```python
from build123d import *

# Parameters (mm, degrees)
BASE_PLATE_SKETCH_W        = 100
BASE_PLATE_SKETCH_H        = 70
BASE_PLATE_100X70X12_DEPTH = 6
RAISED_PAD_SKETCH_W        = 94
RAISED_PAD_SKETCH_H        = 60
RAISED_PAD_94X60X4_DEPTH   = 4
PAD_CUT_1_DEPTH            = 2
PAD_CUT_2_DEPTH            = 2
PAD_CUT_3_DEPTH            = 2


with BuildPart() as part:
    # Base Plate Sketch → Base Plate 100x70x12 (new, symmetric)
    with BuildSketch(Plane.XY):
        Rectangle(BASE_PLATE_SKETCH_W, BASE_PLATE_SKETCH_H)
    extrude(amount=BASE_PLATE_100X70X12_DEPTH, both=True)

    # Raised Pad Sketch → Raised Pad 94x60x4 (add)
    with BuildSketch(Plane(origin=(0, 0, -6), x_dir=(-1, 0, 0), z_dir=(0, 0, -1))):
        Rectangle(RAISED_PAD_SKETCH_W, RAISED_PAD_SKETCH_H)
    extrude(amount=RAISED_PAD_94X60X4_DEPTH)

    # Pad Cut 1 Sketch → Pad Cut 1 (cut, symmetric)
    with BuildSketch(Plane(origin=(0, 0, -10), x_dir=(-1, 0, 0), z_dir=(0, 0, -1))):
        with BuildLine():
            Line((47, -23), (47, 23))
            Line((47, 23), (41, 23))
            ThreePointArc((41, 23), (37.464466094, 21.535533906), (36, 18))
            Line((36, 18), (36, 11.5))
            ThreePointArc((36, 11.5), (32.388712156, 0), (36, -11.5))
            Line((36, -11.5), (36, -18))
            ThreePointArc((36, -18), (37.464466094, -21.535533906), (41, -23))
            Line((41, -23), (47, -23))
        make_face()
    extrude(amount=PAD_CUT_1_DEPTH, both=True, mode=Mode.SUBTRACT)

    # Pad Cut 2 Sketch → Pad Cut 2 (cut, symmetric)
    with BuildSketch(Plane(origin=(0, 0, -10), x_dir=(-1, 0, 0), z_dir=(0, 0, -1))):
        with BuildLine():
            Line((-47, -6), (-39, -6))
            Line((-39, -6), (-39, -15))
            ThreePointArc((-39, -15), (-37.535533906, -18.535533906), (-34, -20))
            Line((-34, -20), (-30, -20))
            ThreePointArc((-30, -20), (-26.464466094, -18.535533906), (-25, -15))
            Line((-25, -15), (-25, -6))
            Line((-25, -6), (-22.017780858, -6.01060535))
            ThreePointArc((-22.017780858, -6.01060535), (-18.470758176, -4.552451776), (-17, -1.010636966))
            Line((-17, -1.010636966), (-17, 1))
            ThreePointArc((-17, 1), (-18.464466094, 4.535533906), (-22, 6))
            Line((-22, 6), (-25, 6))
            Line((-25, 6), (-25, 15))
            ThreePointArc((-25, 15), (-26.464466094, 18.535533906), (-30, 20))
            Line((-30, 20), (-34, 20))
            ThreePointArc((-34, 20), (-37.535533906, 18.535533906), (-39, 15))
            Line((-39, 15), (-39, 6))
            Line((-39, 6), (-47, 6))
            Line((-47, 6), (-47, -6))
        make_face()
    extrude(amount=PAD_CUT_2_DEPTH, both=True, mode=Mode.SUBTRACT)

    # Pad Cut 3 Sketch → Pad Cut 3 (cut, symmetric)
    with BuildSketch(Plane(origin=(0, 0, -10), x_dir=(-1, 0, 0), z_dir=(0, 0, -1))):
        with BuildLine():
            ThreePointArc((-10, 5.000015487), (-15.000015487, 0), (-10, -5.000015487))
            ThreePointArc((-10, -5.000015487), (-8.529332614, -8.524177957), (-5.000015487, -9.982431809))
            ThreePointArc((-5.000015487, -9.982431809), (0, -14.982447295), (5.000015487, -9.982431809))
            ThreePointArc((5.000015487, -9.982431809), (8.529332614, -8.524177957), (10, -5.000015487))
            ThreePointArc((10, -5.000015487), (15.000015487, 0), (10, 5.000015487))
            ThreePointArc((10, 5.000015487), (8.529332614, 8.524177957), (5.000015487, 9.982431809))
            ThreePointArc((5.000015487, 9.982431809), (0, 14.982447295), (-5.000015487, 9.982431809))
            ThreePointArc((-5.000015487, 9.982431809), (-8.529332614, 8.524177957), (-10, 5.000015487))
        make_face()
    extrude(amount=PAD_CUT_3_DEPTH, both=True, mode=Mode.SUBTRACT)


solid = part.part
```
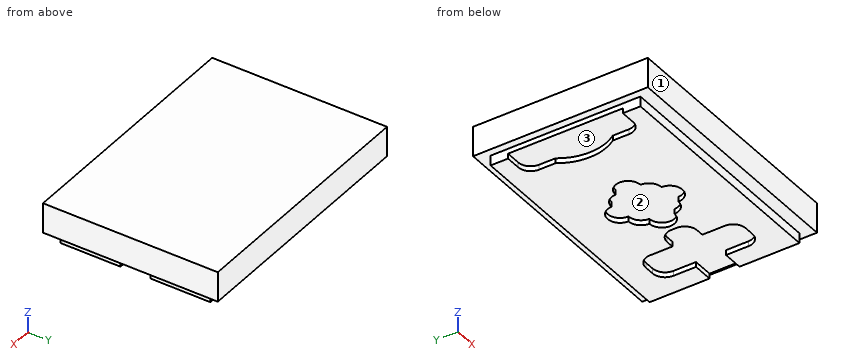
Verification items for the finished model (mm, model axes). Face numbers are marked on the shaded views. A direction names the side the tool comes from. Give positions to 0.01 mm unless a question says otherwise; leave off trailing zeros. Loops run counter-clockwise (first coordinate to the right, second up) from the corner with the lowest first, then second, coordinate; pieces in that order, holes last. Notation, with made-up numbers: M -39,-33.5 L -31,-33.5 A26 cw -31,3.5 Z; hole C -33,18.25 d3. An arc over 180 degrees is marked long. One line per question, with ' | ' between items.
Item 1: Thickness scan on line 1 (Y direction, x = 33, z = -8.25); line 2 (Z direction, x = -46, y = -19); line 3 (X direction, y = 11, z = -6.25). Record the ranges inside material, lowest first. Write a range as [from, to].
Completed:
line 1: y = [-30, -20], [20, 30] | line 2: z = [-8, 6] | line 3: x = [-47, 47]
Item 2: Depth check by flat-ended pin: P1, Ø2, axis at y = -9.5, z = -8.5, coming from the +X side; P2, Ø1.6, axis at x = 33, z = -9.5, coming from the +Y side; P3, Ø1.6, axis at x = 44.5, z = -9, coming from the -Y side. Enter the tip coordinate at first touch or a pass-through.
Completed:
P1: stops at x = 47 | P2: stops at y = 30 | P3: stops at y = -30
Item 3: Section check D-D, the plane x = 19. Record the cut outline in (y, z).
Completed:
outline: M -35,-6 L -30,-6 L -30,-10 L -5.01,-10 L -5.01,-8 L 5,-8 L 5,-10 L 30,-10 L 30,-6 L 35,-6 L 35,6 L -35,6 Z
Item 4: Section check A-A, the plane y = 28. Record the cut outline in (x, z).
Completed:
outline: M -50,-6 L -47,-6 L -47,-10 L 47,-10 L 47,-6 L 50,-6 L 50,6 L -50,6 Z
Item 5: Tool access check on the marked faces 1, 2 and 3. Record the directions out of +Z, -Z, +X, -X, +Y, -Y that give a thin tool (end or side, any length) a straight path to the whole face; none if there is none.
Completed:
face 1: +Z, -Z, +X, -X, -Y | face 2: -Z | face 3: -Z, -X
Item 6: Section check B-B, the plane x = -19. Record the cut outline in (y, z), plus the area to 3 significant figures.
Completed:
outline: M -35,-6 L -30,-6 L -30,-10 L 30,-10 L 30,-6 L 35,-6 L 35,6 L -35,6 Z | area: 1,080 mm^2
Item 7: Section check C-C, the plane y = 0. Record the cut outline in (x, z), plus the area to 3 significant figures.
Completed:
outline: M -50,-6 L -47,-6 L -47,-8 L -32.39,-8 L -32.39,-10 L -15,-10 L -15,-8 L 15,-8 L 15,-10 L 17,-10 L 17,-8 L 47,-8 L 47,-6 L 50,-6 L 50,6 L -50,6 Z | area: 1,430 mm^2
